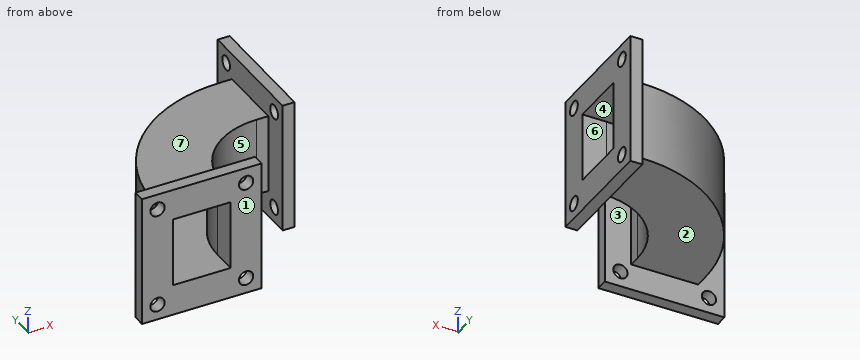
```python
from build123d import *

# Parameters (mm, degrees)
INLET_FLANGE_SKETCH_W    = 55
INLET_FLANGE_SKETCH_H    = 50
INLET_FLANGE_SKETCH_R    = 3
INLET_FLANGE_SKETCH_W_2  = 29
INLET_FLANGE_SKETCH_H_2  = 24
INLET_FLANGE_5MM_DEPTH   = 5
OUTLET_FLANGE_SKETCH_W   = 50
OUTLET_FLANGE_SKETCH_H   = 55
OUTLET_FLANGE_SKETCH_R   = 3
OUTLET_FLANGE_SKETCH_W_2 = 24
OUTLET_FLANGE_SKETCH_H_2 = 29
OUTLET_FLANGE_5MM_DEPTH  = 5
BEND_PROFILE_SKETCH_W    = 28
BEND_PROFILE_SKETCH_H    = 33
BEND_PROFILE_SKETCH_W_2  = 24
BEND_PROFILE_SKETCH_H_2  = 29


with BuildPart() as part:
    # Inlet Flange Sketch → Inlet Flange 5mm (new body)
    with BuildSketch(Plane(origin=(0, 0, 0), x_dir=(0, 0, -1), z_dir=(1, 0, 0))):
        Rectangle(INLET_FLANGE_SKETCH_W, INLET_FLANGE_SKETCH_H)
        with Locations((-21, 18.5)):
            Circle(INLET_FLANGE_SKETCH_R, mode=Mode.SUBTRACT)
        with Locations((21, 18.5)):
            Circle(INLET_FLANGE_SKETCH_R, mode=Mode.SUBTRACT)
        with Locations((21, -18.5)):
            Circle(INLET_FLANGE_SKETCH_R, mode=Mode.SUBTRACT)
        with Locations((-21, -18.5)):
            Circle(INLET_FLANGE_SKETCH_R, mode=Mode.SUBTRACT)
        Rectangle(INLET_FLANGE_SKETCH_W_2, INLET_FLANGE_SKETCH_H_2, mode=Mode.SUBTRACT)
    extrude(amount=INLET_FLANGE_5MM_DEPTH)



with BuildPart() as body_2:
    # Outlet Flange Sketch → Outlet Flange 5mm (new body)
    with BuildSketch(Plane(origin=(0, -50, 0), x_dir=(1, 0, 0), z_dir=(0, 1, 0))):
        with Locations((-50, 0)):
            Rectangle(OUTLET_FLANGE_SKETCH_W, OUTLET_FLANGE_SKETCH_H)
        with Locations(Location((-68.5, 21, 0), (0, 0, 270))):
            Circle(OUTLET_FLANGE_SKETCH_R, mode=Mode.SUBTRACT)
        with Locations(Location((-31.5, 21, 0), (0, 0, 270))):
            Circle(OUTLET_FLANGE_SKETCH_R, mode=Mode.SUBTRACT)
        with Locations(Location((-31.5, -21, 0), (0, 0, 270))):
            Circle(OUTLET_FLANGE_SKETCH_R, mode=Mode.SUBTRACT)
        with Locations(Location((-68.5, -21, 0), (0, 0, 270))):
            Circle(OUTLET_FLANGE_SKETCH_R, mode=Mode.SUBTRACT)
        with Locations((-50, 0)):
            Rectangle(OUTLET_FLANGE_SKETCH_W_2, OUTLET_FLANGE_SKETCH_H_2, mode=Mode.SUBTRACT)
    extrude(amount=-OUTLET_FLANGE_5MM_DEPTH)


with BuildPart() as part_1:
    add(part.part)

    add(body_2.part)  # Elbow Bend Wall 2mm merges body 2
    # Elbow Bend Wall 2mm: sweep along a path in Bend Path R45 Sketch
    with BuildLine(Plane.XY) as elbow_bend_wall_2mm_path:
        Line((-50, -50), (-50, -45))
        ThreePointArc((-50, -45), (-36.819805153, -13.180194847), (-5, 0))
        Line((-5, 0), (0, 0))
    # Bend Profile Sketch → Elbow Bend Wall 2mm (sweep)
    with BuildSketch(Plane(origin=(0, -50, 0), x_dir=(1, 0, 0), z_dir=(0, 1, 0))):
        with Locations((-50, 0)):
            Rectangle(BEND_PROFILE_SKETCH_W, BEND_PROFILE_SKETCH_H)
        with Locations((-50, 0)):
            Rectangle(BEND_PROFILE_SKETCH_W_2, BEND_PROFILE_SKETCH_H_2, mode=Mode.SUBTRACT)
    sweep(path=elbow_bend_wall_2mm_path.line)


solid = part_1.part
```
For this review, take the finished solid that the model builds, in its own axes (mm). Face numbers are marked on the shaded views. A direction names the side the tool comes from. Give positions to 0.01 mm unless a question says otherwise; leave off trailing zeros. Order: outer loops, then holes, each group sorted by start corner. A loop starts at its lowest first (then second) coordinate and runs counter-clockwise, first axis right, second up.
1) Insertion check: pin 1 (9.5 mm diameter, centred on x = -68.5, z = 21, fed in from +Y); pin 2 (2.5 mm diameter, centred on x = 1.5, z = -10, fed in from -Y); pin 3 (5 mm diameter, centred on x = -25.5, y = 2.5, fed in from -Z); pin 4 (5.5 mm diameter, centred on x = -68.5, z = -21, fed in from -Y). Each pin has a flat end and moves straight along its axis. Give the tip position at first contact, or say it passes through.
2) Take a section at D-D (y = -18.5). Give the boundary of the cut face in (x, z).
3) The part is to be moulded in two halves that separate along Y. For the marked faces 1, 2 and 3, say which applies: released by +Y, released by -Y, zero draft, split by the parting line, or undercut.
4) Wall thickness on line 1 (Y direction, x = 2.95, z = 21); line 2 (X direction, y = -51.5, z = -21); line 3 (Y direction, x = 1, z = 11.5): over which ranges is each line inside the solid? List them lowest first.
5) Take a section at C-C (z = -12). Give the boundary of the cut face in (x, y).
6) Take a section at A-A (x = -68.5). Give the boundary of the cut face in (y, z), then the cut area to 3 significant figures.
7) Take a section at B-B (y = 18.5). Give the boundary of the cut face in (x, z).
8) For the marked faces 4, 5, 6 and 7, list the 3-axis set-ups (+Z, -Z, +X, -X, +Y, -Y) from which the entire face can be reached by the end or side of a thin tool; tool diameter is ignored.
Derived:
1. pin 1: stops at y = -50
1. pin 2: stops at y = -25
1. pin 3: stops at z = -16.5
1. pin 4: passes through
2. outline: (-57.71, -16.5) - (-21.09, -16.5) - (-21.09, 16.5) - (-57.71, 16.5) - close; (0, -27.5) - (5, -27.5) - (5, -24) - (0, -24) - close; (0, -18) - (5, -18) - (5, 18) - (0, 18) - close; (0, 24) - (5, 24) - (5, 27.5) - (0, 27.5) - close; hole (-55.47, -14.5) - (-24.67, -14.5) - (-24.67, 14.5) - (-55.47, 14.5) - close
3. face 1: released by -Y
3. face 2: zero draft
3. face 3: undercut
4. line 1: y = -25 to -21.5, -15.5 to 15.5, 21.5 to 25
4. line 2: x = -75 to -71.5, -65.5 to -34.5, -28.5 to -25
4. line 3: y = -25 to -12, 12 to 25
5. outline: (-75, -55) - (-62, -55) - (-62, -45) arc R57 cw to (-5, 12) - (5, 12) - (5, 25) - (0, 25) - (0, 14) - (-5, 14) arc R59 ccw to (-64, -45) - (-64, -50) - (-75, -50) - close; (-38, -55) - (-25, -55) - (-25, -50) - (-36, -50) - (-36, -45) arc R31 cw to (-5, -14) - (0, -14) - (0, -25) - (5, -25) - (5, -12) - (-5, -12) arc R33 ccw to (-38, -45) - close
6. outline: (-55, -27.5) - (-50, -27.5) - (-50, -24) - (-55, -24) - close; (-55, -18) - (-50, -18) - (-50, 18) - (-55, 18) - close; (-55, 24) - (-50, 24) - (-50, 27.5) - (-55, 27.5) - close
6. area: 215 mm2
7. outline: (0, -27.5) - (5, -27.5) - (5, -24) - (0, -24) - close; (0, -18) - (5, -18) - (5, 18) - (0, 18) - close; (0, 24) - (5, 24) - (5, 27.5) - (0, 27.5) - close
8. face 4: none
8. face 5: +Z, -Z
8. face 6: +X
8. face 7: +Z, -X, +Y
